from build123d import *

# Parameters (mm, degrees)
BOSS_EXTRUDE1_DEPTH            = 8
CHAMFER1_SIZE                  = 0.2
CUT_EXTRUDE1_REACH             = 23.401
SKETCH4_R                      = 1.75
CUT_EXTRUDE1_DIRECTION_2_DEPTH = 22.400934559


with BuildPart() as part:
    # Sketch2 → Boss-Extrude1 (new body)
    with BuildSketch(Plane.XY):
        Polygon((-10.793974552, 0), (-8.793974552, 0), (-8.793974552, 15), (-4.793974552, 15), (-4.793974552, 0), (4.206025448, 0), (4.206025448, -4), (-10.793974552, -4), align=None)
    extrude(amount=BOSS_EXTRUDE1_DEPTH)

    # Chamfer1
    chamfer1_edges = [part.edges().sort_by_distance(p)[0] for p in [
        (-0.293974552, 0, 0),
        (4.206025448, -2, 0),
        (-3.293974552, -4, 0),
        (-10.793974552, -2, 0),
        (4.206025448, -2, 8),
        (-10.793974552, 0, 4),
        (-8.793974552, 0, 4),
        (-8.793974552, 15, 4),
        (-4.793974552, 15, 4),
        (-4.793974552, 0, 4),
        (4.206025448, 0, 4),
        (-10.793974552, -4, 4),
        (-0.293974552, 0, 8),
        (-4.793974552, 7.5, 8),
        (-6.793974552, 15, 8),
        (-8.793974552, 7.5, 8),
        (-9.793974552, 0, 8),
        (-10.793974552, -2, 8),
        (-9.793974552, 0, 0),
        (-3.293974552, -4, 8),
        (-8.793974552, 7.5, 0),
        (-6.793974552, 15, 0),
        (-4.793974552, 7.5, 0),
    ]]
    chamfer(chamfer1_edges, length=CHAMFER1_SIZE)

    # Sketch4 → Cut-Extrude1 (cut, up to next)
    with BuildSketch(Plane.ZY.offset(8.793974552), mode=Mode.PRIVATE) as cut_extrude1_sk1:
        with Locations(Location((4, 11, 0), (0, 0, 180))):
            Circle(SKETCH4_R)
    cut_extrude1_tool1 = extrude(cut_extrude1_sk1.sketch, amount=-CUT_EXTRUDE1_REACH, mode=Mode.PRIVATE) & part.part
    # Sketch4 → Cut-Extrude1 (cut, up to next)
    with BuildSketch(Plane.ZY.offset(8.793974552), mode=Mode.PRIVATE) as cut_extrude1_sk2:
        with Locations(Location((4, 3.5, 0), (0, 0, 180))):
            Circle(SKETCH4_R)
    cut_extrude1_tool2 = extrude(cut_extrude1_sk2.sketch, amount=-CUT_EXTRUDE1_REACH, mode=Mode.PRIVATE) & part.part
    add(cut_extrude1_tool1.solids().sort_by_distance((-8.793975, 11, 4))[0], mode=Mode.SUBTRACT)
    add(cut_extrude1_tool2.solids().sort_by_distance((-8.793975, 3.5, 4))[0], mode=Mode.SUBTRACT)

    # Sketch4 → Cut-Extrude1 direction 2 (cut)
    with BuildSketch(Plane.ZY.offset(8.793974552)):
        with Locations(Location((4, 11, 0), (0, 0, 180))):
            Circle(SKETCH4_R)
        with Locations(Location((4, 3.5, 0), (0, 0, 180))):
            Circle(SKETCH4_R)
    extrude(amount=CUT_EXTRUDE1_DIRECTION_2_DEPTH, mode=Mode.SUBTRACT)


solid = part.part
Input: part model. Units: mm. Frame: model coordinates. A direction names the side the tool comes from. Coordinates: 2 decimals unless noted, no trailing zeros. Loops run counter-clockwise (first coordinate to the right, second up) from the corner with the lowest first, then second, coordinate; pieces in that order, holes last.
Q1. Cut plane D-D (y = 13). Output: boundary loops of the cut face in (x, z).
Q2. Contact query for flat-ended pins moving along their axis: pin 1 (4 mm diameter, centred on y = 6, z = 4, fed in from -X); pin 2 (0.5 mm diameter, centred on x = -10, z = 5.5, fed in from +Y); pin 3 (4 mm diameter, centred on y = 4.5, z = 2.5, fed in from +X). Output: stop coordinate, or through.
Q3. Cut plane A-A (y = 3.5). Output: boundary loops of the cut face in (x, z), then the cut area to 3 significant figures.
Q4. Draft query along Z for faces 1 (the face through (-10.794, -2, 4)), 2 (the face through (-6, 1, 0)), 3 (the face through (-6.82, 9.82, 5.29)), 4 (the face through (-6.82, 4.56, 5.39)). Return one class per face: +Z half, -Z half, draft (parallel to the pull), parting line (faces both ways), or undercut.
Q5. Cut plane C-C (x = -0.75). Output: boundary loops of the cut face in (y, z).
Q6. Set-up query: faces 5 (the face through (-7, 15, 4)), 6 (the face through (-8.794, 7, 4)), 7 (the face through (-4.794, 8, 4)). Return all of +Z, -Z, +X, -X, +Y, -Y with unobstructed straight access to the full face (end or side cutting, diameter ignored); none if empty.
Q7. Material intervals for line 1 (Y direction, x = -6.7, z = 4); line 2 (Z direction, x = -7.05, y = 11); line 3 (Y direction, x = -3, z = 4), sorted ascending.
Q8. Cut plane B-B (z = 4). Output: boundary loops of the cut face in (x, y), then the cut area to 3 significant figures.
Working result:
1. outline: (-8.79, 0.2) - (-8.59, 0) - (-4.99, 0) - (-4.79, 0.2) - (-4.79, 7.8) - (-4.99, 8) - (-8.59, 8) - (-8.79, 7.8) - close
2. pin 1: stops at x = -8.79
2. pin 2: stops at y = 0
2. pin 3: stops at x = -4.79
3. outline: (-8.79, 0.2) - (-8.59, 0) - (-4.99, 0) - (-4.79, 0.2) - (-4.79, 2.25) - (-8.79, 2.25) - close; (-8.79, 5.75) - (-4.79, 5.75) - (-4.79, 7.8) - (-4.99, 8) - (-8.59, 8) - (-8.79, 7.8) - close
3. area: 17.9 mm2
4. face 1: draft
4. face 2: -Z half
4. face 3: undercut
4. face 4: undercut
5. outline: (-4, 0.2) - (-3.8, 0) - (-0.2, 0) - (0, 0.2) - (0, 7.8) - (-0.2, 8) - (-3.8, 8) - (-4, 7.8) - close
6. face 5: +Z, -Z, +X, -X, +Y
6. face 6: +Z, -Z, -X, +Y
6. face 7: +Z, -Z, +X, +Y
7. line 1: y = -4 to 1.75, 5.25 to 9.25, 12.75 to 15
7. line 2: z = 0 to 2.25, 5.75 to 8
7. line 3: y = -4 to 0
8. outline: (-10.79, -3.8) - (-10.59, -4) - (4.21, -4) - (4.21, -0.2) - (4.01, 0) - (-4.59, 0) - (-4.79, 0.2) - (-4.79, 1.75) - (-8.79, 1.75) - (-8.79, 0.2) - (-8.99, 0) - (-10.59, 0) - (-10.79, -0.2) - close; (-8.79, 5.25) - (-4.79, 5.25) - (-4.79, 9.25) - (-8.79, 9.25) - close; (-8.79, 12.75) - (-4.79, 12.75) - (-4.79, 14.8) - (-4.99, 15) - (-8.59, 15) - (-8.79, 14.8) - close
8. area: 91.9 mm2
